from build123d import *

# Parameters (mm, degrees)
SKETCH16_R     = 3.4
SKETCH16_R_2   = 3
MEMBER_1_DEPTH = 1467


with BuildPart() as part:
    # Sketch16 → Member 1 (new body)
    with BuildSketch(Plane(origin=(0, 0, 0), x_dir=(-1, 0, 0), z_dir=(0, 1, 0))):
        with BuildLine():
            Line((-5.1, 20), (-5.1, 19.5))
            Line((-5.1, 19.5), (-4.1, 19.5))
            Line((-4.1, 19.5), (-4.1, 17))
            Line((-4.1, 17), (-6.1, 17))
            Line((-6.1, 17), (-6.1, 18))
            Line((-6.1, 18), (-10.3, 18))
            Line((-10.3, 18), (-10.3, 12))
            Line((-10.3, 12), (-6, 7.7))
            Line((-6, 7.7), (6, 7.7))
            Line((6, 7.7), (10.3, 12))
            Line((10.3, 12), (10.3, 18))
            Line((10.3, 18), (6.1, 18))
            Line((6.1, 18), (6.1, 17))
            Line((6.1, 17), (4.1, 17))
            Line((4.1, 17), (4.1, 19.5))
            Line((4.1, 19.5), (5.1, 19.5))
            Line((5.1, 19.5), (5.1, 20))
            Line((5.1, 20), (15.5, 20))
            ThreePointArc((15.5, 20), (18.681980515, 18.681980515), (20, 15.5))
            Line((20, 15.5), (20, 5.1))
            Line((20, 5.1), (19.5, 5.1))
            Line((19.5, 5.1), (19.5, 4.1))
            Line((19.5, 4.1), (17, 4.1))
            Line((17, 4.1), (17, 6.1))
            Line((17, 6.1), (18, 6.1))
            Line((18, 6.1), (18, 10.3))
            Line((18, 10.3), (12, 10.3))
            Line((12, 10.3), (7.7, 6))
            Line((7.7, 6), (7.7, -6))
            Line((7.7, -6), (12, -10.3))
            Line((12, -10.3), (18, -10.3))
            Line((18, -10.3), (18, -6.1))
            Line((18, -6.1), (17, -6.1))
            Line((17, -6.1), (17, -4.1))
            Line((17, -4.1), (19.5, -4.1))
            Line((19.5, -4.1), (19.5, -5.1))
            Line((19.5, -5.1), (20, -5.1))
            Line((20, -5.1), (20, -15.5))
            ThreePointArc((20, -15.5), (18.681980515, -18.681980515), (15.5, -20))
            Line((15.5, -20), (5.1, -20))
            Line((5.1, -20), (5.1, -19.5))
            Line((5.1, -19.5), (4.1, -19.5))
            Line((4.1, -19.5), (4.1, -17))
            Line((4.1, -17), (6.1, -17))
            Line((6.1, -17), (6.1, -18))
            Line((6.1, -18), (10.3, -18))
            Line((10.3, -18), (10.3, -12))
            Line((10.3, -12), (6, -7.7))
            Line((6, -7.7), (-6, -7.7))
            Line((-6, -7.7), (-10.3, -12))
            Line((-10.3, -12), (-10.3, -18))
            Line((-10.3, -18), (-6.1, -18))
            Line((-6.1, -18), (-6.1, -17))
            Line((-6.1, -17), (-4.1, -17))
            Line((-4.1, -17), (-4.1, -19.5))
            Line((-4.1, -19.5), (-5.1, -19.5))
            Line((-5.1, -19.5), (-5.1, -20))
            Line((-5.1, -20), (-15.5, -20))
            ThreePointArc((-15.5, -20), (-18.681980515, -18.681980515), (-20, -15.5))
            Line((-20, -15.5), (-20, -5.1))
            Line((-20, -5.1), (-19.5, -5.1))
            Line((-19.5, -5.1), (-19.5, -4.1))
            Line((-19.5, -4.1), (-17, -4.1))
            Line((-17, -4.1), (-17, -6.1))
            Line((-17, -6.1), (-18, -6.1))
            Line((-18, -6.1), (-18, -10.3))
            Line((-18, -10.3), (-12, -10.3))
            Line((-12, -10.3), (-7.7, -6))
            Line((-7.7, -6), (-7.7, 6))
            Line((-7.7, 6), (-12, 10.3))
            Line((-12, 10.3), (-18, 10.3))
            Line((-18, 10.3), (-18, 6.1))
            Line((-18, 6.1), (-17, 6.1))
            Line((-17, 6.1), (-17, 4.1))
            Line((-17, 4.1), (-19.5, 4.1))
            Line((-19.5, 4.1), (-19.5, 5.1))
            Line((-19.5, 5.1), (-20, 5.1))
            Line((-20, 5.1), (-20, 15.5))
            ThreePointArc((-20, 15.5), (-18.681980515, 18.681980515), (-15.5, 20))
            Line((-15.5, 20), (-5.1, 20))
        make_face()
        Circle(SKETCH16_R, mode=Mode.SUBTRACT)
        with Locations((-15.556349186, 15.556349186)):
            Circle(SKETCH16_R_2, mode=Mode.SUBTRACT)
        with Locations((15.556349186, 15.556349186)):
            Circle(SKETCH16_R_2, mode=Mode.SUBTRACT)
        with Locations((15.556349186, -15.556349186)):
            Circle(SKETCH16_R_2, mode=Mode.SUBTRACT)
        with Locations((-15.556349186, -15.556349186)):
            Circle(SKETCH16_R_2, mode=Mode.SUBTRACT)
    extrude(amount=MEMBER_1_DEPTH)


solid = part.part
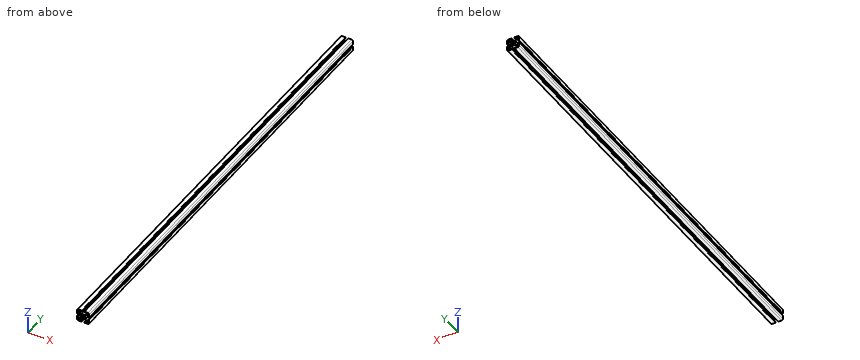
Part model, mm, in its own coordinate system. Round coordinates to 2 decimals unless told otherwise and drop trailing zeros. Use CSV: the item, a comma, the result in double quotes.
Item 1: Slice it at A-A, the plane y = 158. Count the separate pieces of the cut face and the enclosed holes in it, then the cut area to 3 significant figures.
Results list:
separate pieces,"1"
enclosed holes,"5"
area,"605 mm²"
Item 2: Wall check: L1, parallel to Z at x = -16.5, y = 1170; L2, parallel to X at y = 154, z = -4.5. Give the ranges that are in metal, low to high.
Results list:
L1,"z = -19.89 to -18.4, -12.71 to -10.3, 10.3 to 12.71, 18.4 to 19.89"
L2,"x = -19.5 to -17, -7.7 to 7.7, 17 to 19.5"
Item 3: Flat gauge pins, fed straight in: P1, Ø0.8, axis at x = 17.5, y = 744.5, coming from the -Z side; P2, Ø0.8, axis at x = -4.5, y = 822.5, coming from the +Z side. Where does each tip first touch, or does it go through?
Results list:
P1,"stops at z = -19.71"
P2,"stops at z = 19.5"
